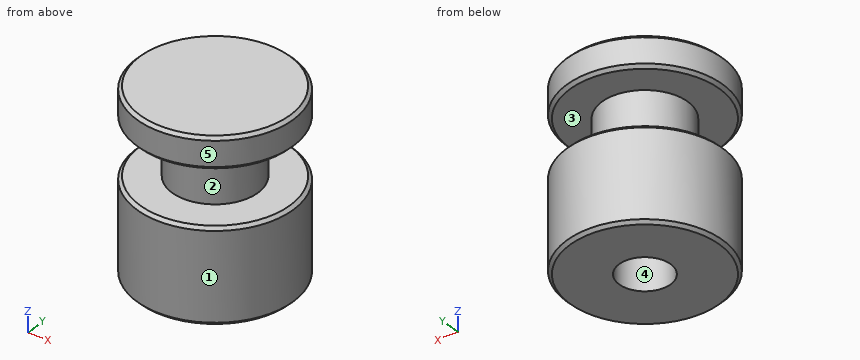
from build123d import *

# Parameters (mm, degrees)
SKETCH1_R             = 5
BOSS_EXTRUDE1_DEPTH   = 6
SKETCH2_R             = 2.75
BOSS_EXTRUDE2_DEPTH   = 3.5
SKETCH3_R             = 5
BOSS_EXTRUDE3_DEPTH   = 2
M4_TAPPED_HOLE1_D     = 3.3
M4_TAPPED_HOLE1_DEPTH = 8
M4_TAPPED_HOLE1_TIP   = 0.991420021
CHAMFER1_SIZE         = 0.2


with BuildPart() as part:
    # Sketch1 → Boss-Extrude1 (new body)
    with BuildSketch(Plane.XY):
        Circle(SKETCH1_R)
    extrude(amount=BOSS_EXTRUDE1_DEPTH)

    # Sketch2 → Boss-Extrude2 (add)
    with BuildSketch(Plane.XY.offset(6)):
        Circle(SKETCH2_R)
    extrude(amount=BOSS_EXTRUDE2_DEPTH)

    # Sketch3 → Boss-Extrude3 (add)
    with BuildSketch(Plane.XY.offset(9.5)):
        Circle(SKETCH3_R)
    extrude(amount=BOSS_EXTRUDE3_DEPTH)

    # M4 tapped hole1
    with Locations(Plane(origin=(0, 0, 0), x_dir=(-1, 0, 0), z_dir=(0, 0, -1))):
        with Locations((0, 0)):
            Hole(M4_TAPPED_HOLE1_D / 2, depth=M4_TAPPED_HOLE1_DEPTH)
            with Locations((0, 0, -(M4_TAPPED_HOLE1_DEPTH + M4_TAPPED_HOLE1_TIP / 2))):  # 118° drill point
                Cone(0, M4_TAPPED_HOLE1_D / 2, M4_TAPPED_HOLE1_TIP, mode=Mode.SUBTRACT)

    # Chamfer1
    chamfer1_edges = [part.edges().sort_by_distance(p)[0] for p in [
        (-5, 0, 0),
        (-5, 0, 6),
        (-5, 0, 9.5),
        (-5, 0, 11.5),
    ]]
    chamfer(chamfer1_edges, length=CHAMFER1_SIZE)


solid = part.part
Source: CAD feature listing. Evaluate the final solid. Frame: model axes, mm. Face numbers are marked on the shaded views. A direction names the side the tool comes from. Round coordinates to 2 decimals unless told otherwise and drop trailing zeros. Write each loop counter-clockwise with the first axis right and the second up, starting at its lowest first coordinate (ties: lowest second). Pieces come first, ordered by that corner, then holes. Notation, with made-up numbers: M 40.5,24.25 L 68.5,24.25 A25 ccw 68.5,56.25 Z; hole C 58.5,11 d7. An arc over 180 degrees is marked long. One line per item, written item: value. Start each with the question number.
Item 1: Set-up query: the marked faces 1 and 2. Return all of +Z, -Z, +X, -X, +Y, -Y with unobstructed straight access to the full face (end or side cutting, diameter ignored); none if empty.
Item 2: Pin query (flat end, axial travel): pin 1 (1 mm diameter, centred on y = 1.5, z = 5, fed in from -X); pin 2 (1.5 mm diameter, centred on x = 2.5, z = 5.5, fed in from -Y); pin 3 (1 mm diameter, centred on y = 1.5, z = 7, fed in from +X). Return the tip coordinate at first contact, or that it passes through.
Item 3: Mould query, pull axis Y, two halves, no side actions, for the marked faces 3, 4 and 5. Classes: pulls with the +Y half, pulls with the -Y half, needs draft (parallel to the pull), parting line crosses it, or undercut.
Item 4: Section query A-A (z = 2.75). Return the cut outline in (x, y), plus the area to 3 significant figures.
Item 5: Section query B-B (z = 10.5). Return the cut outline in (x, y), plus the area to 3 significant figures.
Item 6: Section query C-C (z = 6.5). Return the cut outline in (x, y), plus the area to 3 significant figures.
Item 7: Ray query, L1, parallel to Z at x = -1.5, y = -4; L2, parallel to Y at x = 0, z = 2; L3, parallel to Z at x = 3.5, y = -3.5. Return the intervals inside material, ascending. Write a range as from..to.
Result set:
1. face 1: +Z, -Z
1. face 2: none
2. pin 1: stops at x = -4.9
2. pin 2: stops at y = -4.68
2. pin 3: stops at x = 2.56
3. face 3: needs draft
3. face 4: undercut
3. face 5: parting line crosses it
4. outline: C 0,0 d10; hole C 0,0 d3.3
4. area: 70.0 mm²
5. outline: C 0,0 d10
5. area: 78.5 mm²
6. outline: C 0,0 d5.5; hole C 0,0 d3.3
6. area: 15.2 mm²
7. L1: z = 0..6, 9.5..11.5
7. L2: y = -5..-1.65, 1.65..5
7. L3: z = 0.15..5.85, 9.65..11.35
